```python
from build123d import *

# Parameters (mm, degrees)
CUT_EXTRUDE_1_DEPTH = 2.5


with BuildPart() as part:
    # 草图1 → 旋转1 (revolve)
    with BuildSketch(Plane.XY, mode=Mode.PRIVATE) as revolve_1_sk:
        with BuildLine():
            Line((17, 0), (17, -2.0095))
            Line((17, -2.0095), (16.5095, -2.5))
            Line((16.5095, -2.5), (5, -2.5))
            Line((5, -2.5), (5, -4.25))
            Line((5, -4.25), (0.3, -4.25))
            ThreePointArc((0.3, -4.25), (0.087867966, -4.162132034), (0, -3.95))
            Line((0, -3.95), (0, 0))
            Line((0, 0), (17, 0))
        make_face()
    revolve(revolve_1_sk.sketch.rotate(Axis((0, 0, 0), (1, 0, 0)), 90), axis=Axis((0, 0, 0), (1, 0, 0)))

    # 草图2 → 切除-拉伸1 (cut)
    with BuildSketch(Plane(origin=(0, 0, 0), x_dir=(0, 0, -1), z_dir=(1, 0, 0))):
        Polygon((-1.7, -0.981495458), (0, -1.962990915), (1.7, -0.981495458), (1.7, 0.981495458), (0, 1.962990915), (-1.7, 0.981495458), align=None)
    extrude(amount=CUT_EXTRUDE_1_DEPTH, mode=Mode.SUBTRACT)


solid = part.part
```
Source: CAD feature listing. Evaluate the final solid. Frame: model axes, mm. A direction names the side the tool comes from. Coordinates: 2 decimals unless noted, no trailing zeros. Loops run counter-clockwise (first coordinate to the right, second up) from the corner with the lowest first, then second, coordinate; pieces in that order, holes last. Notation, with made-up numbers: (39.25, -14) -> (49.25, -14) arc R22 cw to (49.25, 14) -> close; hole circle Ø7 at (-37, 5.25). An arc over 180 degrees is marked (long way). One line per item, written item: value. Start each with the question number.
Q1. Mould query, pull axis Z, two halves, no side actions, for faces 4 (the face through (0, 0, -2)), 5 (the face through (1.2, 1.5, 0.8)), 6 (the face through (10.7, 0.1, 2.5)). Classes: pulls with the +Z half, pulls with the -Z half, needs draft (parallel to the pull), parting line crosses it, or undercut.
Q2. Section query A-A, the plane x = 1.75. Return the cut outline in (y, z), and give its area (3 significant figures).
Q3. Contact query for flat-ended pins moving along their axis: P1, Ø5, axis at x = 14, z = -1, coming from the +Y side; P2, Ø2, axis at x = 8.5, z = 1.5, coming from the +Y side; P3, Ø1.5, axis at x = 2.5, z = -2, coming from the -Y side. Output: stop coordinate, or through.
Q4. Section query D-D, the plane x = 3.5. Return the cut outline in (y, z), and give its area (3 significant figures).
Q5. Set-up query: faces 1 (the face through (5, -2, 2)), 2 (the face through (2.617, 4.214, 0.553)), 3 (the face through (1.2, -1.5, -0.8)). Return all of +Z, -Z, +X, -X, +Y, -Y with unobstructed straight access to the full face (end or side cutting, diameter ignored); none if empty.
Q6. Line query: line 1 along Z through (x, y) = (0.5, -0.5); line 2 along Z through (x, y) = (2.25, 1); line 3 along Y through (x, z) = (7.5, 0). Output: solid intervals per line, ascending.
Q7. Section query C-C, the plane x = 7. Return the cut outline in (y, z).
Q8. Section query B-B, the plane y = 0. Return the cut outline in (x, z).
Results:
1. face 4: needs draft
1. face 5: undercut
1. face 6: parting line crosses it
2. outline: circle Ø8.5 at (0, 0); hole (-1.96, 0) -> (-0.98, -1.7) -> (0.98, -1.7) -> (1.96, 0) -> (0.98, 1.7) -> (-0.98, 1.7) -> close
2. area: 46.7 mm^2
3. P1: y = 2.5
3. P2: y = 2.45
3. P3: y = -4.06
4. outline: circle Ø8.5 at (0, 0)
4. area: 56.7 mm^2
5. face 1: +X
5. face 2: +X, -X
5. face 3: -X
6. line 1: -4.22 to -1.7, 1.7 to 4.22
6. line 2: -4.13 to -1.67, 1.67 to 4.13
6. line 3: -2.5 to 2.5
7. outline: circle Ø5 at (0, 0)
8. outline: (0, -3.95) arc R0.3 ccw to (0.3, -4.25) -> (5, -4.25) -> (5, -2.5) -> (16.51, -2.5) -> (17, -2.01) -> (17, 2.01) -> (16.51, 2.5) -> (5, 2.5) -> (5, 4.25) -> (0.3, 4.25) arc R0.3 ccw to (0, 3.95) -> (0, 1.7) -> (2.5, 1.7) -> (2.5, -1.7) -> (0, -1.7) -> close
